```python
from build123d import *

# Parameters (mm, degrees)
CUT_EXTRUDE_1_DEPTH = 6


with BuildPart() as part:
    # Sketch 1 → Revolve 1 (revolve)
    with BuildSketch(Plane.XY, mode=Mode.PRIVATE) as revolve_1_sk:
        Polygon((0, 10), (-8.1, 10), (-8.1, 0), (-5, 0), (-5, -75), (0, -75), align=None)
    revolve(revolve_1_sk.sketch.rotate(Axis((0, 11.322033898, 0), (0, -1, 0)), 270), axis=Axis((0, 11.322033898, 0), (0, -1, 0)))

    # Sketch 2 → Cut-Extrude 1 (cut)
    with BuildSketch(Plane(origin=(0, 10, 0), x_dir=(1, 0, 0), z_dir=(0, 1, 0))):
        Polygon((0, 4.618802154), (-4, 2.309401077), (-4, -2.309401077), (0, -4.618802154), (4, -2.309401077), (4, 2.309401077), align=None)
    extrude(amount=-CUT_EXTRUDE_1_DEPTH, mode=Mode.SUBTRACT)


solid = part.part
```
Here's how the part is built. I have some questions about the finished solid (model axes, mm). A direction names the side the tool comes from. Give positions to 0.01 mm unless a question says otherwise; leave off trailing zeros. Write each loop counter-clockwise with the first axis right and the second up, starting at its lowest first coordinate (ties: lowest second). Pieces come first, ordered by that corner, then holes.
(1) Imagine slicing it at A-A, the plane z = 0. Write out the boundary of the cut face in (x, y).
Output values:
outline: (-8.1, 0) - (-5, 0) - (-5, -75) - (5, -75) - (5, 0) - (8.1, 0) - (8.1, 10) - (4, 10) - (4, 4) - (-4, 4) - (-4, 10) - (-8.1, 10) - close
(2) Imagine slicing it at D-D, the plane z = -7. Write out the boundary of the cut face in (x, y).
Output values:
outline: (-4.08, 0) - (4.08, 0) - (4.08, 10) - (-4.08, 10) - close
(3) Will these pins go through, and if not, where does the flat tip stop? pin 1 (5 mm diameter, centred on x = -2.5, y = -64.5, fed in from +Z); pin 2 (1.4 mm diameter, centred on y = 6, z = -1, fed in from -X); pin 3 (2 mm diameter, centred on y = -23, z = 0, fed in from +X).
Output values:
pin 1: stops at z = 5
pin 2: stops at x = -8.09
pin 3: stops at x = 5
(4) On a 3-axis mill with a long thin cutter (end or side, diameter ignored), from which of +Z, -Z, +X, -X, +Y, -Y can I reach the whole of each face in a straight line? I mean faces 1 (the face through (2, 10, 4)), 2 (the face through (4.88, -38.02, -1.08)), 3 (the face through (-4, 7, 0)). Say none if no direction works.
Output values:
face 1: +Z, -Z, +X, -X, +Y
face 2: -Y
face 3: +Y
(5) Thinking about a two-plate mould opening in Z: for faces 4 (the face through (4, 7, 0)), 5 (the face through (0, 4, 0)), 6 (the face through (7.186, 4.93, 3.738)), 7 (the face through (5.3, 0, -0.1)), which applies, pulls with the +Z half, pulls with the -Z half, needs draft (parallel to the pull), parting line crosses it, or undercut?
Output values:
face 4: undercut
face 5: undercut
face 6: parting line crosses it
face 7: needs draft
(6) Imagine slicing it at C-C, the plane y = -54. Write out the boundary of the cut face in (x, z).
Output values:
outline: circle Ø10 at (0, 0)
(7) Imagine slicing it at B-B, the plane x = 2.25. Write out the boundary of the cut face in (y, z), and give its area (3 significant figures).
Output values:
outline: (-75, -4.47) - (0, -4.47) - (0, -7.78) - (10, -7.78) - (10, -3.32) - (4, -3.32) - (4, 3.32) - (10, 3.32) - (10, 7.78) - (0, 7.78) - (0, 4.47) - (-75, 4.47) - close
area: 786 mm2
(8) If I drill on L1, parallel to Y at x = 6.25, z = -1.75; L2, parallel to Y at x = -3, z = 0.5; L3, parallel to Z at x = 3, y = -55, over which ranges is the centre line in solid material (lowest first)?
Output values:
L1: y = 0 to 10
L2: y = -75 to 4
L3: z = -4 to 4
